Input: part model. Units: mm. Frame: model coordinates. Face numbers are marked on the shaded views. Round coordinates to 2 decimals unless told otherwise and drop trailing zeros. Order: outer loops, then holes, each group sorted by start corner. A loop starts at its lowest first (then second) coordinate and runs counter-clockwise, first axis right, second up. Notation, with made-up numbers: M 88,52.5 L 128,52.5 A23 cw 128,61.5 Z; hole C 24.5,-8.5 d9. An arc over 180 degrees is marked long. One line per question, with ' | ' between items.
```python
from build123d import *

# Parameters (mm, degrees)
SKETCH1_R           = 775
SKETCH1_R_2         = 30
SKETCH1_R_3         = 13
BOSS_EXTRUDE1_DEPTH = 25
M16_TAPPED_HOLE1_D  = 14
SKETCH4_R           = 760
CUT_EXTRUDE1_DEPTH  = 3


with BuildPart() as part:
    # Sketch1 → Boss-Extrude1 (new body)
    with BuildSketch(Plane(origin=(0, 0, 0), x_dir=(1, 0, 0), z_dir=(0, 1, 0))):
        with Locations(Location((0, 0, 0), (0, 0, 270))):
            Circle(SKETCH1_R)
        with Locations(Location((0, 663, 0), (0, 0, 270))):
            Circle(SKETCH1_R_2, mode=Mode.SUBTRACT)
        with Locations(Location((0, -663, 0), (0, 0, 90))):
            Circle(SKETCH1_R_2, mode=Mode.SUBTRACT)
        with Locations(Location((0, 737, 0), (0, 0, 270))):
            Circle(SKETCH1_R_3, mode=Mode.SUBTRACT)
        with Locations(Location((143.781567326, 722.838751657, 0), (0, 0, 270))):
            Circle(SKETCH1_R_3, mode=Mode.SUBTRACT)
        with Locations(Location((282.037689653, 680.899215461, 0), (0, 0, 270))):
            Circle(SKETCH1_R_3, mode=Mode.SUBTRACT)
        with Locations(Location((409.455261735, 612.793104267, 0), (0, 0, 270))):
            Circle(SKETCH1_R_3, mode=Mode.SUBTRACT)
        with Locations(Location((521.137697734, 521.137697734, 0), (0, 0, 270))):
            Circle(SKETCH1_R_3, mode=Mode.SUBTRACT)
        with Locations(Location((612.793104267, 409.455261735, 0), (0, 0, 270))):
            Circle(SKETCH1_R_3, mode=Mode.SUBTRACT)
        with Locations(Location((680.899215461, 282.037689653, 0), (0, 0, 270))):
            Circle(SKETCH1_R_3, mode=Mode.SUBTRACT)
        with Locations(Location((722.838751657, 143.781567326, 0), (0, 0, 270))):
            Circle(SKETCH1_R_3, mode=Mode.SUBTRACT)
        with Locations(Location((737, 0, 0), (0, 0, 270))):
            Circle(SKETCH1_R_3, mode=Mode.SUBTRACT)
        with Locations(Location((722.838751657, -143.781567326, 0), (0, 0, 270))):
            Circle(SKETCH1_R_3, mode=Mode.SUBTRACT)
        with Locations(Location((680.899215461, -282.037689653, 0), (0, 0, 270))):
            Circle(SKETCH1_R_3, mode=Mode.SUBTRACT)
        with Locations(Location((612.793104267, -409.455261735, 0), (0, 0, 270))):
            Circle(SKETCH1_R_3, mode=Mode.SUBTRACT)
        with Locations(Location((521.137697734, -521.137697734, 0), (0, 0, 270))):
            Circle(SKETCH1_R_3, mode=Mode.SUBTRACT)
        with Locations(Location((409.455261735, -612.793104267, 0), (0, 0, 270))):
            Circle(SKETCH1_R_3, mode=Mode.SUBTRACT)
        with Locations(Location((282.037689653, -680.899215461, 0), (0, 0, 270))):
            Circle(SKETCH1_R_3, mode=Mode.SUBTRACT)
        with Locations(Location((143.781567326, -722.838751657, 0), (0, 0, 270))):
            Circle(SKETCH1_R_3, mode=Mode.SUBTRACT)
        with Locations(Location((0, -737, 0), (0, 0, 270))):
            Circle(SKETCH1_R_3, mode=Mode.SUBTRACT)
        with Locations(Location((-143.781567326, -722.838751657, 0), (0, 0, 270))):
            Circle(SKETCH1_R_3, mode=Mode.SUBTRACT)
        with Locations(Location((-282.037689653, -680.899215461, 0), (0, 0, 270))):
            Circle(SKETCH1_R_3, mode=Mode.SUBTRACT)
        with Locations(Location((-409.455261735, -612.793104267, 0), (0, 0, 270))):
            Circle(SKETCH1_R_3, mode=Mode.SUBTRACT)
        with Locations(Location((-521.137697734, -521.137697734, 0), (0, 0, 270))):
            Circle(SKETCH1_R_3, mode=Mode.SUBTRACT)
        with Locations(Location((-612.793104267, -409.455261735, 0), (0, 0, 270))):
            Circle(SKETCH1_R_3, mode=Mode.SUBTRACT)
        with Locations(Location((-680.899215461, -282.037689653, 0), (0, 0, 270))):
            Circle(SKETCH1_R_3, mode=Mode.SUBTRACT)
        with Locations(Location((-722.838751657, -143.781567326, 0), (0, 0, 270))):
            Circle(SKETCH1_R_3, mode=Mode.SUBTRACT)
        with Locations(Location((-737, 0, 0), (0, 0, 270))):
            Circle(SKETCH1_R_3, mode=Mode.SUBTRACT)
        with Locations(Location((-722.838751657, 143.781567326, 0), (0, 0, 270))):
            Circle(SKETCH1_R_3, mode=Mode.SUBTRACT)
        with Locations(Location((-680.899215461, 282.037689653, 0), (0, 0, 270))):
            Circle(SKETCH1_R_3, mode=Mode.SUBTRACT)
        with Locations(Location((-612.793104267, 409.455261735, 0), (0, 0, 270))):
            Circle(SKETCH1_R_3, mode=Mode.SUBTRACT)
        with Locations(Location((-521.137697734, 521.137697734, 0), (0, 0, 270))):
            Circle(SKETCH1_R_3, mode=Mode.SUBTRACT)
        with Locations(Location((-409.455261735, 612.793104267, 0), (0, 0, 270))):
            Circle(SKETCH1_R_3, mode=Mode.SUBTRACT)
        with Locations(Location((-282.037689653, 680.899215461, 0), (0, 0, 270))):
            Circle(SKETCH1_R_3, mode=Mode.SUBTRACT)
        with Locations(Location((-143.781567326, 722.838751657, 0), (0, 0, 270))):
            Circle(SKETCH1_R_3, mode=Mode.SUBTRACT)
        with BuildLine():
            Line((225, -425), (-225, -425))
            ThreePointArc((-225, -425), (-366.421356237, -366.421356237), (-425, -225))
            Line((-425, -225), (-425, 225))
            ThreePointArc((-425, 225), (-366.421356237, 366.421356237), (-225, 425))
            Line((-225, 425), (225, 425))
            ThreePointArc((225, 425), (366.421356237, 366.421356237), (425, 225))
            Line((425, 225), (425, -225))
            ThreePointArc((425, -225), (366.421356237, -366.421356237), (225, -425))
        make_face(mode=Mode.SUBTRACT)
    extrude(amount=BOSS_EXTRUDE1_DEPTH)

    # M16 Tapped Hole1 (through all)
    with Locations(Plane(origin=(0, 25, 0), x_dir=(1, 0, 0), z_dir=(0, 1, 0))):
        with Locations((-635.5, -55.5), (-524.5, -55.5), (-524.5, 55.5), (-635.5, 55.5), (635.5, 55.5), (524.5, 55.5), (524.5, -55.5), (635.5, -55.5)):
            Hole(M16_TAPPED_HOLE1_D / 2)

    # Sketch4 → Cut-Extrude1 (cut)
    with BuildSketch(Plane.XZ):
        with Locations(Location((0, 0, 0), (0, 0, 270))):
            Circle(SKETCH4_R)
    extrude(amount=-CUT_EXTRUDE1_DEPTH, mode=Mode.SUBTRACT)


solid = part.part
```
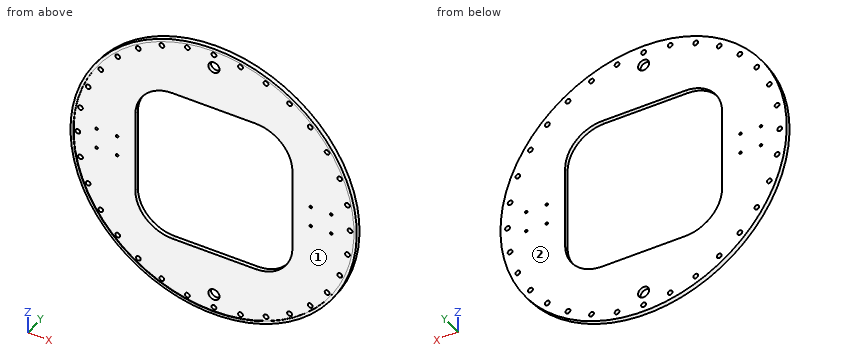
Item 1: Mould query, pull axis X, two halves, no side actions, for the marked faces 1 and 2. Classes: +X half, -X half, draft (parallel to the pull), parting line (faces both ways), or undercut.
Report:
face 1: undercut | face 2: draft
Item 2: Section query B-B, the plane y = 9.25. Give the number of separate pieces and of enclosed holes in the cut face, plus the area to 3 significant figures.
Report:
separate pieces: 1 | enclosed holes: 43 | area: 1,170,000 mm²
Item 3: First-contact query: pin 1 (11 mm diameter, centred on y = 18.5, z = 82, fed in from -X); pin 2 (6 mm diameter, centred on x = 394, y = 3, fed in from +Z); pin 3 (10 mm diameter, centred on x = 136.5, y = 19, fed in from -Z); pin 4 (12.5 mm diameter, centred on x = -524.5, z = 55.5, fed in from -Y). Flat tips, straight axial feed; report the tip coordinate or a pass-through.
Report:
pin 1: x = -771.22 | pin 2: z = 669.14 | pin 3: z = -763.76 | pin 4: through
Item 4: Line query: line 1 along X through (y, z) = (20, -622); line 2 along Z through (x, y) = (635.5, 14.75); line 3 along Z through (x, y) = (154.5, 22.5). Output: solid intervals per line, ascending. Write a range as from..to.
Report:
line 1: -462.32..-418.63, -400.28..400.28, 418.63..462.32 | line 2: -443.58..-62.5, -48.5..48.5, 62.5..443.58 | line 3: -759.44..-730.2, -715.48..-425, 425..715.48, 730.2..759.44
Item 5: Section query A-A, the plane x = -72. Return loops of the section in (y, z), plus the area to 3 significant figures.
Report:
outline: M 0,-771.65 L 25,-771.65 L 25,-425 L 3,-425 L 3,-756.58 L 0,-756.58 Z; M 0,756.58 L 3,756.58 L 3,425 L 25,425 L 25,771.65 L 0,771.65 Z | area: 15,300 mm²
